The listing builds one solid part. Answer for the finished solid, in the listing's coordinates (mm). Face numbers are marked on the shaded views. Coordinates: 2 decimals unless noted, no trailing zeros. Order: outer loops, then holes, each group sorted by start corner. A loop starts at its lowest first (then second) coordinate and runs counter-clockwise, first axis right, second up. Notation, with made-up numbers: (-3.75, 71.5) -> (8.25, 71.5) arc R13 ccw to (8.25, 91.5) -> close; hole circle Ø2 at (65.25, -18). An arc over 180 degrees is marked (long way). Write item = value, one per line. Start each with the question number.
```python
from build123d import *

# Parameters (mm, degrees)
SKETCH_1_R           = 4
SKETCH_1_R_2         = 2
EXTRUDE_1_DEPTH      = 8
EXTRUDE_2_DEPTH      = 12
EXTRUDE_2_DEPTH_BACK = 6
SKETCH_3_R           = 5


with BuildPart() as part:
    # 草图1 → 凸台-拉伸1 (new body)
    with BuildSketch(Plane.XY):
        with Locations((2.360745364, -1.287337305)):
            Circle(SKETCH_1_R)
        with Locations((2.360745364, -1.287337305)):
            Circle(SKETCH_1_R_2, mode=Mode.SUBTRACT)
    extrude(amount=EXTRUDE_1_DEPTH)

    # 草图3 → 凸台-拉伸2 (add, two sides: drawn at the far end of the back side and taken through both)
    with BuildSketch(Plane(origin=(0, 0, 0), x_dir=(1, 0, 0), z_dir=(0, 1, 0)).offset(-EXTRUDE_2_DEPTH_BACK)):
        with Locations(Location((2.360745364, 0, 0), (0, 0, 270))):
            Circle(SKETCH_3_R)
    extrude(amount=EXTRUDE_2_DEPTH + EXTRUDE_2_DEPTH_BACK)


solid = part.part
```
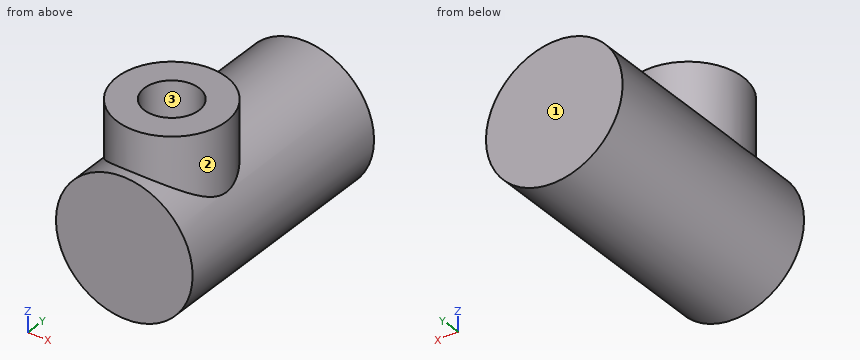
Item 1: Section C-C, the plane y = 5 is taken. Give the vertices of the cut face in (x, z), then the cut area to 3 significant figures.
Item 2: For a pull along Y with two mould halves and no side action, classify the marked faces 1, 2 and 3 as pulls with the +Y half, pulls with the -Y half, needs draft (parallel to the pull), parting line crosses it, or undercut.
Item 3: Section D-D, the plane z = 7 is taken. Give the vertices of the cut face in (x, y).
Item 4: Consider probe 1 along Z at (x, y) = (2.5, 1); probe 2 along X at (y, z) = (4.25, -4); probe 3 along Y at (x, z) = (-0.75, 4). Determine where each line is inside the solid, lowest interval first.
Item 5: Section A-A, the plane x = -1.25 is taken. Give the vertices of the cut face in (y, z), then the cut area to 3 significant figures.
Item 6: Each of these flat-tipped pins is pushed along its axis until it touches: pin 1 (3.5 mm diameter, centred on x = 2.36, y = -1.29, fed in from +Z); pin 2 (1 mm diameter, centred on y = -3.5, z = 2.5, fed in from +X); pin 3 (1.5 mm diameter, centred on y = 0.5, z = 5, fed in from +X). Where does it stop, or does it pass through?
Item 7: Section B-B, the plane z = 3.75 is taken. Give the vertices of the cut face in (x, y).
A:
q1.outline = circle Ø10 at (2.36, 0)
q1.area = 78.5 mm^2
q2.face_1 = pulls with the +Y half
q2.face_2 = parting line crosses it
q2.face_3 = undercut
q3.outline = circle Ø8 at (2.36, -1.29); hole circle Ø4 at (2.36, -1.29)
q4.probe_1 = -5 to 8
q4.probe_2 = -0.64 to 5.36
q4.probe_3 = -3.8 to 1.23
q5.outline = (-6, -3.46) -> (12, -3.46) -> (12, 3.46) -> (0.43, 3.46) -> (0.43, 8) -> (-3.01, 8) -> (-3.01, 3.46) -> (-6, 3.46) -> close
q5.area = 140 mm^2
q6.pin_1 = 5
q6.pin_2 = 6.94
q6.pin_3 = 6.22
q7.outline = (-0.95, -6) -> (5.67, -6) -> (5.67, -3.54) arc R4 ccw to (5.67, 0.96) -> (5.67, 12) -> (-0.95, 12) -> (-0.95, 0.96) arc R4 ccw to (-0.95, -3.54) -> close
